Geometry: final body of the model. Coordinates: model frame, mm. A direction names the side the tool comes from. Give positions to 0.01 mm unless a question says otherwise; leave off trailing zeros. Order: outer loops, then holes, each group sorted by start corner. A loop starts at its lowest first (then second) coordinate and runs counter-clockwise, first axis right, second up. Notation, with made-up numbers: M -38.75,-18.5 L 6.25,-18.5 A26 ccw 6.25,-2.5 Z; hole C 44.5,-27 d6. An arc over 180 degrees is marked long. Use CSV: the item, a comma, the result in double quotes.
```python
from build123d import *

# Parameters (mm, degrees)
SKETCH1_R                                          = 26
SKETCH1_R_2                                        = 21
BOSS_EXTRUDE1_DEPTH                                = 10
SKETCH2_R                                          = 40
BOSS_EXTRUDE2_DEPTH                                = 10
SKETCH3_R                                          = 11
CUT_EXTRUDE1_DEPTH                                 = 10
FILLET1_R                                          = 2
HOLE_SIZE_BASED_HEX_SOCKET_HEAD_CAP_SC_D           = 4.5
HOLE_SIZE_BASED_HEX_SOCKET_HEAD_CAP_SC_CBORE_D     = 8
HOLE_SIZE_BASED_HEX_SOCKET_HEAD_CAP_SC_CBORE_DEPTH = 4.6
CIRPATTERN1_COUNT                                  = 4


with BuildPart() as part:
    # Sketch1 → Boss-Extrude1 (new body)
    with BuildSketch(Plane(origin=(0, 0, 0), x_dir=(1, 0, 0), z_dir=(0, 1, 0))):
        with Locations(Location((0, 0, 0), (0, 0, 270))):
            Circle(SKETCH1_R)
        with Locations(Location((0, 0, 0), (0, 0, 270))):
            Circle(SKETCH1_R_2, mode=Mode.SUBTRACT)
    extrude(amount=BOSS_EXTRUDE1_DEPTH)

    # Sketch2 → Boss-Extrude2 (add)
    with BuildSketch(Plane(origin=(0, 10, 0), x_dir=(1, 0, 0), z_dir=(0, 1, 0))):
        with Locations(Location((0, 0, 0), (0, 0, 270))):
            Circle(SKETCH2_R)
    extrude(amount=BOSS_EXTRUDE2_DEPTH)

    # Sketch3 → Cut-Extrude1 (cut)
    with BuildSketch(Plane.XZ.offset(-10)):
        with Locations(Location((0, 0, 0), (0, 0, 270))):
            Circle(SKETCH3_R)
    extrude(amount=-CUT_EXTRUDE1_DEPTH, mode=Mode.SUBTRACT)

    # Fillet1
    fillet1_edges = [part.edges().sort_by_distance(p)[0] for p in [
        (0, 20, -40),
    ]]
    fillet(fillet1_edges, radius=FILLET1_R)

    # Hole size (%based) hex socket head cap screw type 1 (through all)
    with Locations(Plane(origin=(0, 20, 0), x_dir=(1, 0, 0), z_dir=(0, 1, 0))):
        with Locations((0, 30)):
            hole_size_based_hex_socket_head_cap_sc = CounterBoreHole(HOLE_SIZE_BASED_HEX_SOCKET_HEAD_CAP_SC_D / 2, HOLE_SIZE_BASED_HEX_SOCKET_HEAD_CAP_SC_CBORE_D / 2, HOLE_SIZE_BASED_HEX_SOCKET_HEAD_CAP_SC_CBORE_DEPTH)

    # CirPattern1: Hole size (%based) hex socket head cap screw type 1 ×4 about axis
    cirpattern1_axis = Axis((0, 0, 0), (0, 1, 0))
    for i in range(1, CIRPATTERN1_COUNT):
        add(hole_size_based_hex_socket_head_cap_sc.rotate(cirpattern1_axis, i * 360 / CIRPATTERN1_COUNT), mode=Mode.SUBTRACT)


solid = part.part
```
1. Section D-D, the plane y = 8. Return the cut outline in (x, z), plus the area to 3 significant figures.
Answer:
outline,"C 0,0 d52; hole C 0,0 d42"
area,"738 mm2"
2. Section A-A, the plane x = 0. Give the number of separate pieces and of enclosed holes in the cut face, plus the area to 3 significant figures.
Answer:
separate pieces,"4"
enclosed holes,"0"
area,"556 mm2"
3. Section C-C, the plane y = 12.5. Return the cut outline in (x, z), plus the area to 3 significant figures.
Answer:
outline,"C 0,0 d80; hole C -30,0 d4.5; hole C 0,0 d22; hole C 0,-30 d4.5; hole C 0,30 d4.5; hole C 30,0 d4.5"
area,"4,580 mm2"
4. Pull-direction query (X, two-part tool) for faces 1 (the face through (0.521, 17.732, 33.966)), 2 (the face through (21.3, 0, 1.8)), 3 (the face through (-39.05, 13.94, -8.67)); classes: +X half, -X half, draft (parallel to the pull), parting line (faces both ways), or undercut.
Answer:
face 1,"undercut"
face 2,"draft"
face 3,"parting line"
5. Line query: line 1 (X direction, y = 19.25, z = 2.5); line 2 (Y direction, x = 4, z = -29.5); line 3 (Z direction, x = -27, y = 16.5). Output: solid intervals per line, ascending.
Answer:
line 1,"-39.48 to -33.12, -26.88 to -10.71, 10.71 to 26.88, 33.12 to 39.48"
line 2,"10 to 20"
line 3,"-29.51 to -2.65, 2.65 to 29.51"
6. Reachability of faces 4 (the face through (31.52, 12.66, 1.66)), 5 (the face through (-8, 10, 26)), 6 (the face through (-2, 15.4, 28)) from +Z, -Z, +X, -X, +Y, -Y: full face, straight path, thin tool, end or side. Return the list, or none.
Answer:
face 4,"+Y, -Y"
face 5,"-Y"
face 6,"+Y"
7. Pin query (flat end, axial travel): pin 1 Ø10 at (x, z) = (0.5, -7.5) entering from -Y; pin 2 Ø6 at (x, y) = (31.5, 9) entering from +Z; pin 3 Ø5 at (x, z) = (-30, 0) entering from +Y; pin 4 Ø2.5 at (x, z) = (0, -30) entering from +Y. Return the tip coordinate at first contact, or that it passes through.
Answer:
pin 1,"y = 10"
pin 2,"z = 27.89"
pin 3,"y = 15.4"
pin 4,"through"
